For this review, use the dimensioned drawing (mm, ordinates from the lowest corner) and the shaded views. A direction names the side the tool comes from. Round coordinates to 2 decimals unless told otherwise and drop trailing zeros. Write each loop counter-clockwise with the first axis right and the second up, starting at its lowest first coordinate (ties: lowest second). Pieces come first, ordered by that corner, then holes. Notation, with made-up numbers: (74.25, -19) -> (123.25, -19) arc R29 cw to (123.25, 16) -> close; hole circle Ø9 at (6.5, -36). An arc over 180 degrees is marked (long way). Answer as CSV lines item,"result". Start each with the question number.
Item 1: For pin 1 Ø1 at (y, z) = (29, 11) entering from +X; pin 2 Ø1.6 at (x, z) = (29, 10) entering from +Y; pin 3 Ø4 at (x, z) = (23.5, 9.5) entering from +Y, all flat-tipped, find the tip position at first contact; note any pin that passes through.
Item 2: Mouldability with a two-part tool opening along X and no side actions: class the marked faces 1, 2, 3 and 4 as +X half, -X half, draft (parallel to the pull), parting line (faces both ways), or undercut.
Item 3: Take a section at B-B on z = 5.25. Give the boundary of the cut face in (x, y).
Item 4: Take a section at A-A on x = 15.5. Give the boundary of the cut face in (y, z) (1 decimal).
Item 5: Machinability: for the marked faces 5, 6 and 7, which of the approach directions +Z, -Z, +X, -X, +Y, -Y give a long, thin tool a straight path to every point of the face, cutting with its end or side? Answer none if there is none.
Item 6: Wall thickness on probe 1 along Z at (x, y) = (16, 26.25); probe 2 along Y at (x, z) = (9.75, 6.75) (1 decimal); probe 3 along X at (y, z) = (4.5, 9.5) (1 decimal): over which ranges is each line inside the solid? List them lowest first. Write a range as from..to.
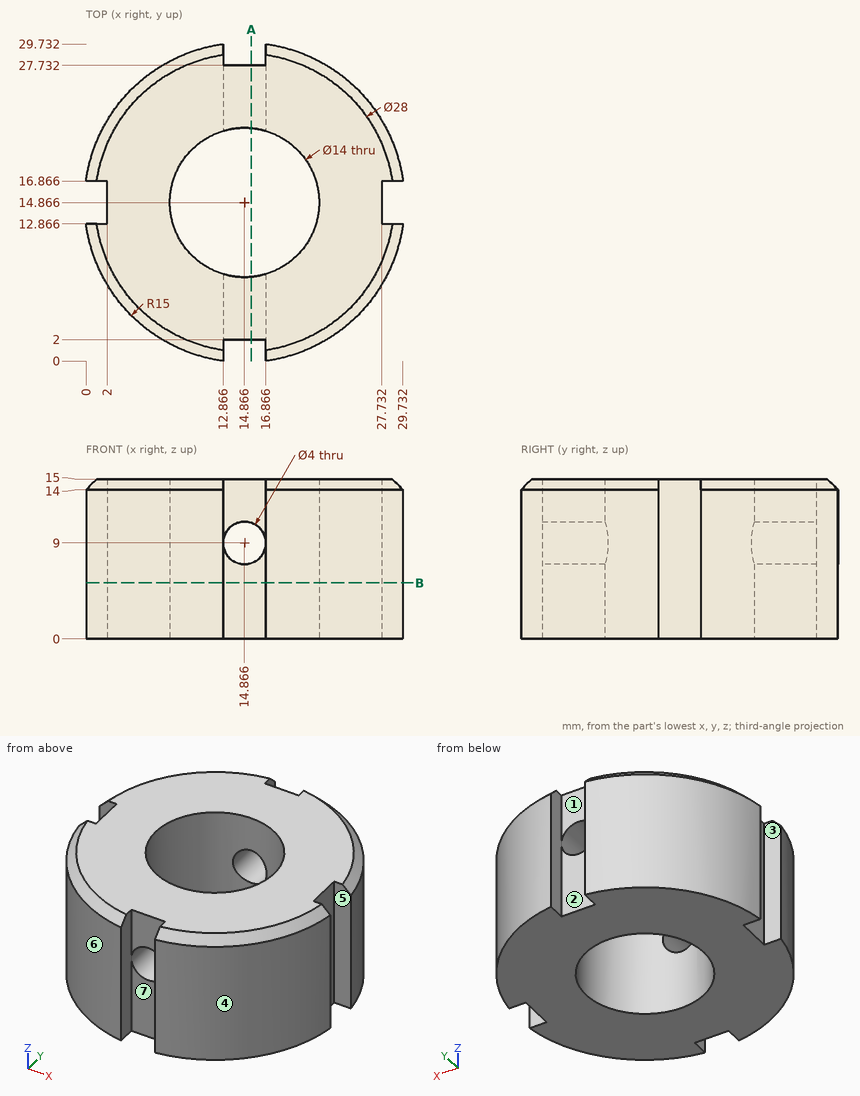
Output values:
1,pin 1,"stops at x = 21.12"
1,pin 2,"stops at y = 21.74"
1,pin 3,"stops at y = 28.32"
2,face 1,"undercut"
2,face 2,"undercut"
2,face 3,"draft"
2,face 4,"+X half"
3,outline,"(0, 12.87) arc R15 ccw to (12.87, 0) -> (12.87, 2) -> (16.87, 2) -> (16.87, 0) arc R15 ccw to (29.73, 12.87) -> (27.73, 12.87) -> (27.73, 16.87) -> (29.73, 16.87) arc R15 ccw to (16.87, 29.73) -> (16.87, 27.73) -> (12.87, 27.73) -> (12.87, 29.73) arc R15 ccw to (0, 16.87) -> (2, 16.87) -> (2, 12.87) -> close; hole circle Ø14 at (14.87, 14.87)"
4,outline,"(2, 0) -> (7.9, 0) -> (7.9, 7.1) -> (2, 7.1) -> close; (2, 10.9) -> (7.9, 10.9) -> (7.9, 15) -> (2, 15) -> close; (21.8, 0) -> (27.7, 0) -> (27.7, 7.1) -> (21.8, 7.1) -> close; (21.8, 10.9) -> (27.7, 10.9) -> (27.7, 15) -> (21.8, 15) -> close"
5,face 5,"+Z, -Z, +X"
5,face 6,"+Z, -Z, -X, -Y"
5,face 7,"+Z, -Z, -Y"
6,probe 1,"z = 0..7.35, 10.65..15"
6,probe 2,"y = 0.8..10.1, 19.6..29"
6,probe 3,"x = 4..12.9, 16.8..25.7"
